from build123d import *

# Parameters (mm, degrees)
SKETCH_1_R          = 3.5
EXTRUDE_1_DEPTH     = 4
CUT_EXTRUDE_1_DEPTH = 2
FILLET_1_R          = 0.2
SKETCH_5_R          = 2
EXTRUDE_2_DEPTH     = 18
CHAMFER_2_SIZE      = 0.39


with BuildPart() as part:
    # 草图1 → 凸台-拉伸1 (new body)
    with BuildSketch(Plane(origin=(0, 0, 0), x_dir=(1, 0, 0), z_dir=(0, 1, 0))):
        with Locations(Location((0, 0, 0), (0, 0, 270))):
            Circle(SKETCH_1_R)
    extrude(amount=EXTRUDE_1_DEPTH)

    # 草图2 → 切除-拉伸1 (cut)
    with BuildSketch(Plane(origin=(0, 4, 0), x_dir=(1, 0, 0), z_dir=(0, 1, 0))):
        Polygon((1.772465326, 0), (0.886232663, 1.535), (-0.886232663, 1.535), (-1.772465326, 0), (-0.886232663, -1.535), (0.886232663, -1.535), align=None)
    extrude(amount=-CUT_EXTRUDE_1_DEPTH, mode=Mode.SUBTRACT)

    # 圆角1
    fillet_1_edges = [part.edges().sort_by_distance(p)[0] for p in [
        (0, 4, -3.5),
    ]]
    fillet(fillet_1_edges, radius=FILLET_1_R)

    # 草图5 → 凸台-拉伸2 (add)
    with BuildSketch(Plane.XZ):
        with Locations(Location((0, 0, 0), (0, 0, 90))):
            Circle(SKETCH_5_R)
    extrude(amount=EXTRUDE_2_DEPTH)

    # 倒角2
    chamfer_2_edges = [part.edges().sort_by_distance(p)[0] for p in [
        (0, -18, -2),
    ]]
    chamfer(chamfer_2_edges, length=CHAMFER_2_SIZE)


solid = part.part
Geometry: final body of the model. Coordinates: model frame, mm. A direction names the side the tool comes from. Round coordinates to 2 decimals unless told otherwise and drop trailing zeros. Loops run counter-clockwise (first coordinate to the right, second up) from the corner with the lowest first, then second, coordinate; pieces in that order, holes last. Notation, with made-up numbers: (-29.5, 15.25) -> (7.5, 15.25) arc R17 cw to (7.5, 30.25) -> close; hole circle Ø5 at (57, 57). An arc over 180 degrees is marked (long way). One line per question, with ' | ' between items. Start each with the question number.
1. Set-up query: faces 1 (the face through (2, -9, 0)), 2 (the face through (2, 4, 1)), 3 (the face through (-1.32, 3.01, -0.78)). Return all of +Z, -Z, +X, -X, +Y, -Y with unobstructed straight access to the full face (end or side cutting, diameter ignored); none if empty.
2. Section B-B on y = -13. Output: boundary loops of the cut face in (x, z), and give its area (3 significant figures).
3. Line query: line 1 along Y through (x, z) = (2, -1); line 2 along Y through (x, z) = (0.5, -0.5); line 3 along X through (y, z) = (-13.75, -0.75). Output: solid intervals per line, ascending. Write a range as [from, to].
4. Section C-C on y = 0.25. Output: boundary loops of the cut face in (x, z), and give its area (3 significant figures).
5. Contact query for flat-ended pins moving along their axis: pin 1 (3 mm diameter, centred on y = -11, z = -0.5, fed in from +X); pin 2 (1 mm diameter, centred on x = 0, y = -13.5, fed in from -Z). Output: stop coordinate, or through.
6. Section A-A on x = 0. Output: boundary loops of the cut face in (y, z) (3 decimals), and give its area (3 significant figures).
7. Mould query, pull axis Z, two halves, no side actions, for faces 4 (the face through (0, -18, 0)), 5 (the face through (0, 2, 0)), 6 (the face through (-3.417, 1.873, -0.759)). Classes: pulls with the +Z half, pulls with the -Z half, needs draft (parallel to the pull), parting line crosses it, or undercut.
Returned:
1) face 1: -Y | face 2: +Z, -Z, +X, -X, +Y | face 3: +Y
2) outline: circle Ø4 at (0, 0) | area: 12.6 mm2
3) line 1: y = [0, 4] | line 2: y = [-18, 2] | line 3: x = [-1.85, 1.85]
4) outline: circle Ø7 at (0, 0) | area: 38.5 mm2
5) pin 1: stops at x = 2 | pin 2: stops at z = -2
6) outline: (-18, -1.61) -> (-17.61, -2) -> (0, -2) -> (0, -3.5) -> (3.8, -3.5) arc R0.2 ccw to (4, -3.3) -> (4, -1.535) -> (2, -1.535) -> (2, 1.535) -> (4, 1.535) -> (4, 3.3) arc R0.2 ccw to (3.8, 3.5) -> (0, 3.5) -> (0, 2) -> (-17.61, 2) -> (-18, 1.61) -> close | area: 93.7 mm2
7) face 4: needs draft | face 5: undercut | face 6: parting line crosses it
